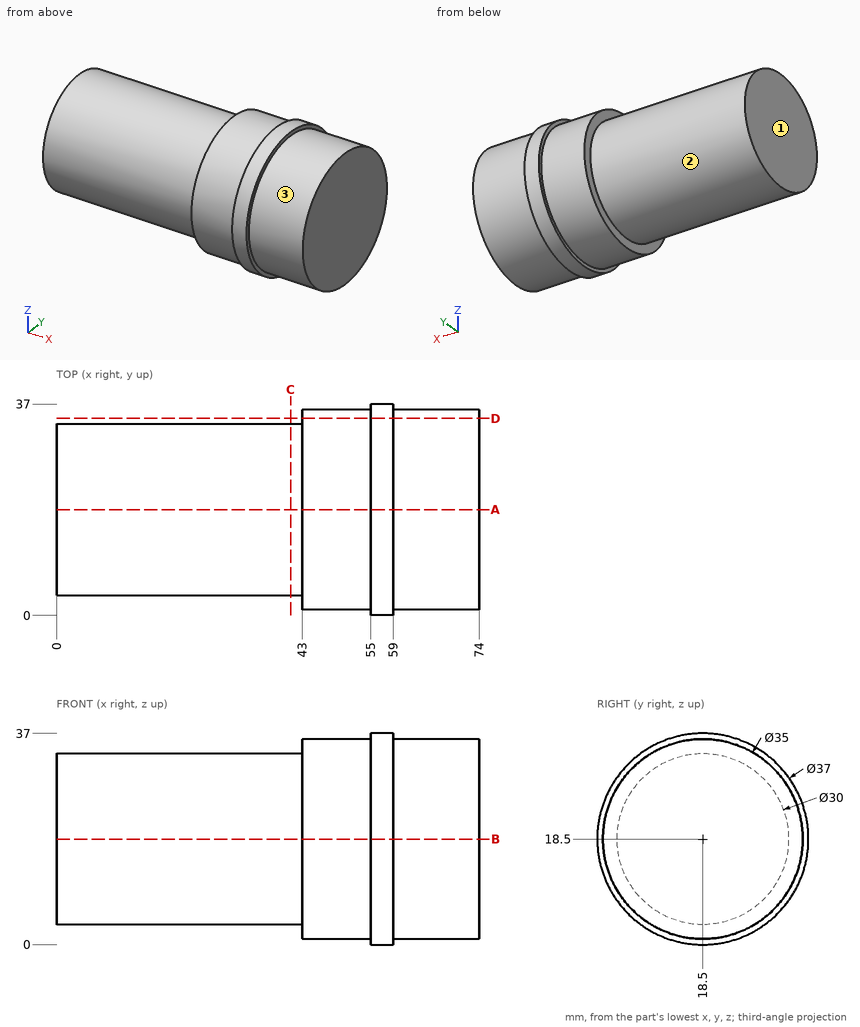
The drawing under review shows one solid part. Ordinate dimensions are in mm from its lowest x, y, z. A direction names the side the tool comes from. Round coordinates to 2 decimals unless told otherwise and drop trailing zeros. Loops run counter-clockwise (first coordinate to the right, second up) from the corner with the lowest first, then second, coordinate; pieces in that order, holes last. Notation, with made-up numbers: (76.25, 61) - (116.25, 61) arc R3 cw to (116.25, 65) - close; hole circle Ø8 at (50, 53). An arc over 180 degrees is marked (long way). One line per question, with ' | ' between items.
Q1. For line 1 along Y through (x, z) = (33.5, 19); line 2 along Z through (x, y) = (44, 27.5); line 3 along X through (y, z) = (14, 3), list the stretches that pass through material, from the lowest coordinate up. Write a range as [from, to].
Taken from the geometry:
line 1: y = [3.51, 33.49] | line 2: z = [3.49, 33.51] | line 3: x = [43, 74]
Q2. Tool access review of the marked faces 1, 2 and 3: name each direction out of +Z, -Z, +X, -X, +Y, -Y from which nothing blocks a thin tool from reaching the whole face with its end or side.
Taken from the geometry:
face 1: +Z, -Z, -X, +Y, -Y | face 2: -X | face 3: +X
Q3. Take a section at A-A (y = 18.5). Give the boundary of the cut face in (x, z), and give its area (3 significant figures).
Taken from the geometry:
outline: (0, 3.5) - (43, 3.5) - (43, 1) - (55, 1) - (55, 0) - (59, 0) - (59, 1) - (74, 1) - (74, 36) - (59, 36) - (59, 37) - (55, 37) - (55, 36) - (43, 36) - (43, 33.5) - (0, 33.5) - close | area: 2,380 mm²
Q4. Take a section at C-C (x = 41). Give the boundary of the cut face in (y, z).
Taken from the geometry:
outline: circle Ø30 at (18.5, 18.5)
Q5. Take a section at D-D (y = 34.5). Give the boundary of the cut face in (x, z), and give its area (3 significant figures).
Taken from the geometry:
outline: (43, 11.41) - (55, 11.41) - (55, 9.21) - (59, 9.21) - (59, 11.41) - (74, 11.41) - (74, 25.59) - (59, 25.59) - (59, 27.79) - (55, 27.79) - (55, 25.59) - (43, 25.59) - close | area: 457 mm²
Q6. For pin 1 (6 mm diameter, centred on x = 46.5, y = 13.5, fed in from -Z); pin 2 (5 mm diameter, centred on x = 29, z = 30.5, fed in from +Y); pin 3 (4 mm diameter, centred on x = 22, z = 24, fed in from +Y); pin 4 (12 mm diameter, centred on y = 4, z = 7.5, fed in from +X), all flat-tipped, find the tip position at first contact; note any pin that passes through.
Taken from the geometry:
pin 1: stops at z = 1.11 | pin 2: stops at y = 30.11 | pin 3: stops at y = 33.09 | pin 4: stops at x = 74
